Source: CAD feature listing. Evaluate the final solid. Frame: model axes, mm. A direction names the side the tool comes from. Give positions to 0.01 mm unless a question says otherwise; leave off trailing zeros. Write each loop counter-clockwise with the first axis right and the second up, starting at its lowest first coordinate (ties: lowest second). Pieces come first, ordered by that corner, then holes. Notation, with made-up numbers: M 35.5,57.25 L 77.5,57.25 A13 cw 77.5,71.25 Z; hole C 38.5,32.5 d10. An arc over 180 degrees is marked long. Answer as a JSON object with one key per item and string values. Group by question number.
```python
from build123d import *

# Parameters (mm, degrees)
CUT_EXTRUDE_3_DEPTH = 352.939625504
CHAMFER_1_SIZE      = 1


with BuildPart() as part:
    # 草图1 → 旋转1 (revolve)
    with BuildSketch(Plane.XY):
        Polygon((0, 0), (0, 10), (17, 10), (17, 9.25), (18.5, 9.25), (18.5, 10), (40.5, 10), (40.5, 12), (60.5, 12), (60.5, 12.5), (110.5, 12.5), (110.5, 19), (116.5, 19), (116.5, 12.5), (122.5, 12.5), (125.5, 10.5), (134.5, 10.5), (134.5, 13), (350.5, 13), (350.5, 0), align=None)
    revolve(axis=Axis((350.5, 0, 0), (-1, 0, 0)))

    # 草图2 → 切除-拉伸3 (cut, through all)
    with BuildSketch(Plane(origin=(0, 6.5, 0), x_dir=(1, 0, 0), z_dir=(0, 1, 0))):
        with BuildLine():
            Line((22, 3), (37.5, 3))
            ThreePointArc((37.5, 3), (40.5, 0), (37.5, -3))
            Line((37.5, -3), (22, -3))
            ThreePointArc((22, -3), (19, 0), (22, 3))
        make_face()
    extrude(amount=CUT_EXTRUDE_3_DEPTH, mode=Mode.SUBTRACT)

    # 倒角1
    chamfer_1_edges = [part.edges().sort_by_distance(p)[0] for p in [
        (350.5, -13, 0),
        (116.5, -19, 0),
        (110.5, -19, 0),
        (40.5, -12, 0),
        (0, -10, 0),
    ]]
    chamfer(chamfer_1_edges, length=CHAMFER_1_SIZE)


solid = part.part
```
(1) Access query for faces 5 (the flat face through (134.5, 9, -6)), 6 (the flat face through (0, 0, 0)), 7 (the cylindrical face through (29.65, -2.17, 9.76)), 8 (the cylindrical face through (113.528, 8.767, 16.856)), 9 (the cylindrical face through (243.505, -10.316, 7.91)). Directions: +Z, -Z, +X, -X, +Y, -Y. A direction counts if a zero-diameter tool reaches every point of the face in a straight line with its end or side. Return the directions, or none.
(2) Section A-A, the plane x = 138.5. Return loops of the section in (y, z), plus the area to 3 significant figures.
(3) Pull-direction query (X, two-part tool) for faces 1 (the flat face through (30, 6.5, 0)), 2 (the flat face through (350.5, 0, 0)), 3 (the cylindrical face through (9.11, -2.17, 9.76)), 4 (the cylindrical face through (17.76, -2.01, 9.03)); classes: pulls with the +X half, pulls with the -X half, needs draft (parallel to the pull), parting line crosses it, or undercut.
(4) Ray query, L1, parallel to X at y = -13, z = -4.5; L2, parallel to Y at x = 104, z = -3.5; L3, parallel to X at y = -4, z = 11. Return the intervals inside material, ascending. Write a range as [from, to].
(5) Contact query for flat-ended pins moving along their axis: pin 1 Ø1.5 at (x, y) = (172, 2) entering from -Z; pin 2 Ø3.5 at (x, y) = (32, 8) entering from +Z; pin 3 Ø1 at (x, z) = (235.5, -2.5) entering from -Y. Output: stop coordinate, or through.
Reported:
{
 "1": {"face 5": "none", "face 6": "+Z, -Z, -X, +Y, -Y", "face 7": "-X", "face 8": "+X, -X", "face 9": "+X"},
 "2": {"outline": "C 0,0 d26", "area": "531 mm2"},
 "3": {"face 1": "undercut", "face 2": "pulls with the +X half", "face 3": "needs draft", "face 4": "undercut"},
 "4": {"L1": "x = [110.5, 116.5]", "L2": "y = [-12, 12]", "L3": "x = [41.2, 123.69], [134.5, 350.5]"},
 "5": {"pin 1": "stops at z = -12.94", "pin 2": "stops at z = 7.81", "pin 3": "stops at y = -12.85"}
}
